Verification items for the finished model (mm, model axes). Face numbers are marked on the shaded views. A direction names the side the tool comes from. Coordinates: 2 decimals unless noted, no trailing zeros. Loops run counter-clockwise (first coordinate to the right, second up) from the corner with the lowest first, then second, coordinate; pieces in that order, holes last.
Q1. Go/stop test with flat-tipped pins: P1, Ø4, axis at x = 2, z = 11.5, coming from the +Y side; P2, Ø4, axis at y = -6, z = 18, coming from the -X side; P3, Ø5, axis at x = 0, y = 2.5, coming from the +Z side; P4, Ø8, axis at x = 3, y = -5.5, coming from the +Z side. Record where each tip stops, or that it passes through.
Q2. Sectioned sample at A-A (z = 15). Enter the section's corners in (x, y).
Q3. Material ranges on probe 1 along Y at (x, z) = (-0.25, 16.25); probe 2 along Y at (x, z) = (-1.5, 5.5); probe 3 along Z at (x, y) = (-7, -1.25), recorded low to high.
Q4. Access from +Z, -Z, +X, -X, +Y, -Y to the whole of each face (thin tool, end or side, straight path). Record for the marked faces 1 and 2.
```python
from build123d import *

# Parameters (mm, degrees)
SKETCH1_R           = 2
BOSS_EXTRUDE1_DEPTH = 10
SKETCH2_R           = 8
BOSS_EXTRUDE2_DEPTH = 8
SKETCH3_R           = 8
SKETCH3_R_2         = 6
CUT_EXTRUDE1_DEPTH  = 3
DOME1_FACE_RADIUS   = 8
DOME1_HEIGHT        = 3
FILLET1_R           = 2


with BuildPart() as part:
    # Sketch1 → Boss-Extrude1 (new body)
    with BuildSketch(Plane.XY):
        Circle(SKETCH1_R)
    extrude(amount=BOSS_EXTRUDE1_DEPTH)

    # Sketch2 → Boss-Extrude2 (add)
    with BuildSketch(Plane.XY.offset(10)):
        Circle(SKETCH2_R)
    extrude(amount=BOSS_EXTRUDE2_DEPTH)

    # Sketch3 → Cut-Extrude1 (cut)
    with BuildSketch(Plane(origin=(0, 0, 10), x_dir=(-1, 0, 0), z_dir=(0, 0, -1))):
        Circle(SKETCH3_R)
        Circle(SKETCH3_R_2, mode=Mode.SUBTRACT)
    extrude(amount=-CUT_EXTRUDE1_DEPTH, mode=Mode.SUBTRACT)

    # Dome1: a dome of height H over a round flat face of radius A is a cap of a sphere of radius (A * A + H * H) / (2 * H)
    dome1_r = (DOME1_FACE_RADIUS * DOME1_FACE_RADIUS + DOME1_HEIGHT * DOME1_HEIGHT) / (2 * DOME1_HEIGHT)
    dome1_base = Plane((0, 0, 18), z_dir=(0, 0, 1))
    with Locations(dome1_base.offset(DOME1_HEIGHT - dome1_r)):
        dome1_ball = Sphere(dome1_r, mode=Mode.PRIVATE)
    add(split(dome1_ball, bisect_by=dome1_base, keep=Keep.TOP, mode=Mode.PRIVATE))

    # Fillet1
    fillet1_edges = [part.edges().sort_by_distance(p)[0] for p in [
        (-8, 0, 18),
    ]]
    fillet(fillet1_edges, radius=FILLET1_R)


solid = part.part
```
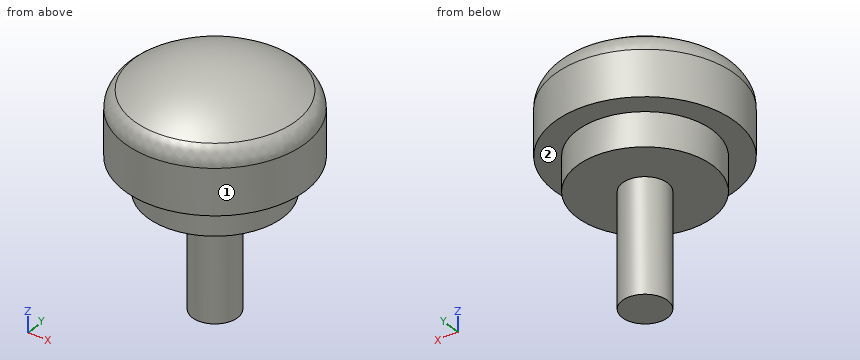
Geometry check:
1. P1: stops at y = 7.97
1. P2: stops at x = -6.84
1. P3: stops at z = 21
1. P4: stops at z = 20.79
2. outline: circle Ø16 at (0, 0)
3. probe 1: y = -8 to 8
3. probe 2: y = -1.32 to 1.32
3. probe 3: z = 13 to 18.71
4. face 1: +Z, -Z
4. face 2: -Z
